```python
from build123d import *

# Parameters (mm, degrees)
SKETCH_1_R      = 12.5
EXTRUDE_1_DEPTH = 35
SKETCH_3_W      = 1.3
SKETCH_3_H      = 0.55
SKETCH_31_W     = 1.3
SKETCH_31_H     = 0.55
CHAMFER_1_SIZE  = 1


with BuildPart() as part:
    # 草图1 → 凸台-拉伸1 (new, symmetric)
    with BuildSketch(Plane.XY):
        Circle(SKETCH_1_R)
    extrude(amount=EXTRUDE_1_DEPTH, both=True)

    # 草图3 → 切除-旋转1 (revolve, cut)
    with BuildSketch(Plane(origin=(-100, 0, -35), x_dir=(0, 0, 1), z_dir=(0, 1, 0))):
        with Locations((3.35, 87.775)):
            Rectangle(SKETCH_3_W, SKETCH_3_H)
    revolve(axis=Axis((0, 0, -35), (0, 0, 1)), mode=Mode.SUBTRACT)

    # 草图31 → 切除-旋转11 (revolve, cut)
    with BuildSketch(Plane(origin=(100, 0, 35), x_dir=(0, 0, -1), z_dir=(0, 1, 0)), mode=Mode.PRIVATE) as cut_revolve_11_sk:
        with Locations((3.35, 87.775)):
            Rectangle(SKETCH_31_W, SKETCH_31_H)
    revolve(cut_revolve_11_sk.sketch.rotate(Axis((0, 0, 35), (0, 0, -1)), 180), axis=Axis((0, 0, 35), (0, 0, -1)), mode=Mode.SUBTRACT)

    # 倒角1
    chamfer_1_edges = [part.edges().sort_by_distance(p)[0] for p in [
        (-12.5, 0, -35),
        (-12.5, 0, 35),
    ]]
    chamfer(chamfer_1_edges, length=CHAMFER_1_SIZE)


solid = part.part
```
Check sheet for the modelled part. Datum: model origin and axes. Units: mm. A direction names the side the tool comes from. Round coordinates to 2 decimals unless told otherwise and drop trailing zeros. Write each loop counter-clockwise with the first axis right and the second up, starting at its lowest first coordinate (ties: lowest second). Pieces come first, ordered by that corner, then holes. Notation, with made-up numbers: (-31, 53.5) -> (-14, 53.5) arc R14 cw to (-14, 59.5) -> close; hole circle Ø7 at (-38.75, 20). An arc over 180 degrees is marked (long way). One line per question, with ' | ' between items. Start each with the question number.
1. Scan lines: line 1 along Y through (x, z) = (0.25, 10); line 2 along Z through (x, y) = (-8, -8.5); line 3 along X through (y, z) = (-8, -15.5). Record each from-to range of solid material in increasing order. Write a range as from..to.
2. Depth check by flat-ended pin: pin 1 (4 mm diameter, centred on x = -6, z = 3.5, fed in from -Y); pin 2 (4 mm diameter, centred on y = -4, z = 13.5, fed in from +X); pin 3 (4 mm diameter, centred on y = 6, z = -19, fed in from -X). Enter the tip coordinate at first touch or a pass-through.
3. Release check for a two-part mould opening along Z. For faces 1 (the face through (0, 0, -35)), 2 (the face through (11.923, 3.755, 33.162)), 3 (the face through (-11.4, -3.59, -31.64)), 4 (the face through (0, 0, 35)) record: +Z half, -Z half, draft (parallel to the pull), parting line (faces both ways), or undercut.
4. Set-up check for faces 5 (the face through (11.923, 3.755, -33.138)), 6 (the face through (-11.4, 3.59, 31.64)): record each of +Z, -Z, +X, -X, +Y, -Y from which the full face is reachable in a straight line by a thin tool's end or side.
5. Sectioned sample at A-A, the plane z = -17. Record the cut outline in (x, y).
Taken from the geometry:
1) line 1: y = -12.5..12.5 | line 2: z = -34.83..34.83 | line 3: x = -9.6..9.6
2) pin 1: stops at y = -11.84 | pin 2: stops at x = 12.34 | pin 3: stops at x = -11.84
3) face 1: -Z half | face 2: draft | face 3: undercut | face 4: +Z half
4) face 5: +Z, -Z | face 6: none
5) outline: circle Ø25 at (0, 0)
